Can you work these out from the model? Positions are in its coordinate system, mm. A direction names the side the tool comes from. Give positions to 0.01 mm unless a question says otherwise; leave off trailing zeros. Loops run counter-clockwise (first coordinate to the right, second up) from the corner with the lowest first, then second, coordinate; pieces in that order, holes last. Notation, with made-up numbers: (-9.5, -25.75) -> (47.5, -25.75) arc R34 ccw to (47.5, 5.25) -> close; hole circle Ø3 at (1.25, 12). An arc over 180 degrees is marked (long way). Return JSON: item names as keys, results as strings. Group by question number.
Q1. Which directions (+Z, -Z, +X, -X, +Y, -Y) give clear straight access to the entire face, cutting with the end or side of a thin tool? Please do faces 4 (the flat face through (-4.3, -10, 11.9)), 5 (the cylindrical face through (0, 15, 28)).
Q2. Will these pins go through, and if not, where does the flat tip stop? pin 1 (6 mm diameter, centred on y = -15.5, z = 24, fed in from -X); pin 2 (3 mm diameter, centred on y = -9.5, z = 18.5, fed in from +X); pin 3 (12 mm diameter, centred on y = -0.5, z = -13.5, fed in from -X).
Q3. Thinking about a two-plate mould opening in Z: for faces 1 (the cylindrical face through (28, 15, 0)), 2 (the flat face through (19, 20, 19)), 3 (the conical face through (-11.632, -9.169, 22.364)), which applies, pulls with the +Z half, pulls with the -Z half, needs draft (parallel to the pull), parting line crosses it, or undercut?
Q4. I need wall thicknesses on line 1 along Z through (x, y) = (-10.5, 1); line 2 along X through (y, z) = (7, -8); line 3 along X through (y, z) = (15.5, 26.5). Which ranges of each line are inside material? Lowest first, please. Write a range as [from, to].
Q5. Suppose I cut it at B-B, the plane x = 0. Please give me the cut outline in (y, z), and give its area (3 significant figures).
Q6. Suppose I cut it at C-C, the plane y = 17. Please give me the cut outline in (x, z), and give its area (3 significant figures).
Q7. Suppose I cut it at D-D, the plane y = -13. Please give me the cut outline in (x, z).
Q8. Suppose I cut it at A-A, the plane z = 0. Please give me the cut outline in (x, y), and give its area (3 significant figures).
```python
from build123d import *

# Parameters (mm, degrees)
SKETCH2_R          = 12.5
CUT_EXTRUDE1_DEPTH = 10
CUT_EXTRUDE2_DEPTH = 40
CIRPATTERN1_COUNT  = 4


with BuildPart() as part:
    # Sketch1 → Revolve1 (revolve)
    with BuildSketch(Plane.XY, mode=Mode.PRIVATE) as revolve1_sk:
        Polygon((32.5, 20), (22.5, -20), (0, -20), (0, -10), (18.299953358, -10), (25.799953358, 20), align=None)
    revolve(revolve1_sk.sketch.rotate(Axis((0, 20, 0), (0, -1, 0)), 180), axis=Axis((0, 20, 0), (0, -1, 0)))

    # Sketch2 → Cut-Extrude1 (cut)
    with BuildSketch(Plane(origin=(0, -10, 0), x_dir=(1, 0, 0), z_dir=(0, 1, 0))):
        with Locations(Location((0, 0, 0), (0, 0, 180))):
            Circle(SKETCH2_R)
    extrude(amount=-CUT_EXTRUDE1_DEPTH, mode=Mode.SUBTRACT)

    # Sketch4 → Cut-Extrude2 (cut, symmetric)
    with BuildSketch(Plane.XY):
        with BuildLine():
            Line((-5, 20), (5, 20))
            ThreePointArc((5, 20), (0, 15), (-5, 20))
        make_face()
    cut_extrude2 = extrude(amount=CUT_EXTRUDE2_DEPTH, both=True, mode=Mode.SUBTRACT)

    # CirPattern1: Cut-Extrude2 ×4 about axis
    cirpattern1_axis = Axis((0, -20, 0), (0, 1, 0))
    for i in range(1, CIRPATTERN1_COUNT):
        add(cut_extrude2.rotate(cirpattern1_axis, i * 360 / CIRPATTERN1_COUNT), mode=Mode.SUBTRACT)


solid = part.part
```
Ans:
{
 "1": {"face 4": "+Y", "face 5": "+Z, -Z, +Y"},
 "2": {"pin 1": "stops at x = -11.05", "pin 2": "stops at x = 18.59", "pin 3": "stops at x = -26.9"},
 "3": {"face 1": "undercut", "face 2": "needs draft", "face 3": "parting line crosses it"},
 "4": {"line 1": "z = [-25.69, -18.24], [18.24, 25.69]", "line 2": "x = [-28.13, -21.08], [21.08, 28.13]", "line 3": "x = [-16.8, -2.18], [2.18, 16.8]"},
 "5": {"outline": "(-20, -22.5) -> (15, -31.25) -> (15, -24.55) -> (-10, -18.3) -> (-10, -12.5) -> (-20, -12.5) -> close; (-20, 12.5) -> (-10, 12.5) -> (-10, 18.3) -> (15, 24.55) -> (15, 31.25) -> (-20, 22.5) -> close", "area": "560 mm^2"},
 "6": {"outline": "(-31.5, -4) arc R31.75 ccw to (-4, -31.5) -> (-4, -24.73) arc R25.05 cw to (-24.73, -4) -> close; (-31.5, 4) -> (-24.73, 4) arc R25.05 cw to (-4, 24.73) -> (-4, 31.5) arc R31.75 ccw to start; (4, -31.5) arc R31.75 ccw to (31.5, -4) -> (24.73, -4) arc R25.05 cw to (4, -24.73) -> close; (4, 24.73) arc R25.05 cw to (24.73, 4) -> (31.5, 4) arc R31.75 ccw to (4, 31.5) -> close", "area": "980 mm^2"},
 "7": {"outline": "circle Ø48.5 at (0, 0); hole circle Ø25 at (0, 0)"},
 "8": {"outline": "(-31.25, 15) -> (-22.5, -20) -> (-12.5, -20) -> (-12.5, -10) -> (-18.3, -10) -> (-24.55, 15) -> close; (12.5, -20) -> (22.5, -20) -> (31.25, 15) -> (24.55, 15) -> (18.3, -10) -> (12.5, -10) -> close", "area": "560 mm^2"}
}
